```python
from build123d import *

# Parameters (mm, degrees)
SKETCH1_R           = 250
BOSS_EXTRUDE1_DEPTH = 3
SKETCH2_R           = 75
CUT_EXTRUDE1_DEPTH  = 10
CIRPATTERN1_COUNT   = 4
SKETCH3_R           = 3
CUT_EXTRUDE2_DEPTH  = 20
CIRPATTERN2_COUNT   = 6


with BuildPart() as part:
    # Sketch1 → Boss-Extrude1 (new body)
    with BuildSketch(Plane(origin=(0, 0, 0), x_dir=(0, 0, -1), z_dir=(1, 0, 0))):
        Circle(SKETCH1_R)
    extrude(amount=BOSS_EXTRUDE1_DEPTH)

    # Sketch2 → Cut-Extrude1 (cut)
    with BuildSketch(Plane(origin=(3, 0, 0), x_dir=(0, 0, -1), z_dir=(1, 0, 0))):
        with Locations((0, 125)):
            Circle(SKETCH2_R)
    cut_extrude1 = extrude(amount=-CUT_EXTRUDE1_DEPTH, mode=Mode.SUBTRACT)

    # CirPattern1: Cut-Extrude1 ×4 about axis
    cirpattern1_axis = Axis((0, 0, 0), (1, 0, 0))
    for i in range(1, CIRPATTERN1_COUNT):
        add(cut_extrude1.rotate(cirpattern1_axis, i * 360 / CIRPATTERN1_COUNT), mode=Mode.SUBTRACT)

    # Sketch3 → Cut-Extrude2 (cut)
    with BuildSketch(Plane(origin=(3, 0, 0), x_dir=(0, 0, -1), z_dir=(1, 0, 0))):
        with Locations((0, -237.5)):
            Circle(SKETCH3_R)
    cut_extrude2 = extrude(amount=-CUT_EXTRUDE2_DEPTH, mode=Mode.SUBTRACT)

    # CirPattern2: Cut-Extrude2 ×6 about axis
    cirpattern2_axis = Axis((0, 0, 0), (1, 0, 0))
    for i in range(1, CIRPATTERN2_COUNT):
        add(cut_extrude2.rotate(cirpattern2_axis, i * 360 / CIRPATTERN2_COUNT), mode=Mode.SUBTRACT)


solid = part.part
```
Read the model definition and answer for the solid it produces. Units are mm, in the model's axes. Coordinates: 2 decimals unless noted, no trailing zeros. Write each loop counter-clockwise with the first axis right and the second up, starting at its lowest first coordinate (ties: lowest second). Pieces come first, ordered by that corner, then holes. Notation, with made-up numbers: (-22.75, 0.5) - (8.25, 0.5) arc R32 cw to (8.25, 36.5) - close; hole circle Ø4 at (39, 34). An arc over 180 degrees is marked (long way). Answer as a JSON object with one key per item and string values. Group by question number.
1. A cutting plane is placed at A-A (y = 0). Determine the outline of the cut face in (x, z), plus the area to 3 significant figures.
2. Each of these flat-tipped pins is pushed along its axis until it touches: P1, Ø9.5, axis at y = -118.75, z = -205.68, coming from the -X side; P2, Ø3.5, axis at y = 118.75, z = -205.68, coming from the +X side; P3, Ø1, axis at x = 2, y = 85.5, coming from the -Z side. Where does it stop, or does it pass through?
3. A cutting plane is placed at D-D (y = -64). Determine the outline of the cut face in (x, z), plus the area to 3 significant figures.
4. A cutting plane is placed at C-C (y = 88.5). Determine the outline of the cut face in (x, z).
5. Consider L1, parallel to Y at x = 1.1, z = 0; L2, parallel to Z at x = 0.65, y = -118.75; L3, parallel to Z at x = 2.5, y = 15.5. Determine where each line is inside the solid, lowest interval first. Write a range as [from, to].
6. The mould has two halves that part along Y. Classify faces 1 (the cylindrical face through (1.521, 9.764, -199.362)), 2 (the cylindrical face through (1.48, 10.99, 249.76)), 3 (the flat face through (0, 4, 3)), 4 (the cylindrical face through (1.521, 199.362, 9.764)): +Y half, -Y half, draft (parallel to the pull), parting line (faces both ways), or undercut.
7. A cutting plane is placed at B-B (z = -91). Determine the outline of the cut face in (x, y), plus the area to 3 significant figures.
Worked out:
{
 "1": {"outline": "(0, -250) - (3, -250) - (3, -200) - (0, -200) - close; (0, -50) - (3, -50) - (3, 50) - (0, 50) - close; (0, 200) - (3, 200) - (3, 250) - (0, 250) - close", "area": "600 mm²"},
 "2": {"P1": "stops at x = 0", "P2": "passes through", "P3": "stops at z = -235.11"},
 "3": {"outline": "(0, -241.67) - (3, -241.67) - (3, -164.1) - (0, -164.1) - close; (0, -85.9) - (3, -85.9) - (3, -43.63) - (0, -43.63) - close; (0, 43.63) - (3, 43.63) - (3, 85.9) - (0, 85.9) - close; (0, 164.1) - (3, 164.1) - (3, 241.67) - (0, 241.67) - close", "area": "719 mm²"},
 "4": {"outline": "(0, -233.81) - (3, -233.81) - (3, -65.52) - (0, -65.52) - close; (0, 65.52) - (3, 65.52) - (3, 233.81) - (0, 233.81) - close"},
 "5": {"L1": "y = [-250, -240.5], [-234.5, -200], [-50, 50], [200, 234.5], [240.5, 250]", "L2": "z = [-220, -208.68], [-202.68, -74.74], [74.74, 202.68], [208.68, 220]", "L3": "z = [-249.52, -198.38], [-51.62, 51.62], [198.38, 249.52]"},
 "6": {"face 1": "undercut", "face 2": "parting line", "face 3": "draft", "face 4": "undercut"},
 "7": {"outline": "(0, -232.85) - (3, -232.85) - (3, -66.85) - (0, -66.85) - close; (0, 66.85) - (3, 66.85) - (3, 232.85) - (0, 232.85) - close", "area": "996 mm²"}
}
